```python
from build123d import *

# Parameters (mm, degrees)
SKETCH_1_W             = 60
SKETCH_1_H             = 67.5
EXTRUDE_1_DEPTH        = 6
CUT_EXTRUDE_1_DEPTH    = 47.723254382
HOLE_WIZARD_M5_1_D     = 4.2
HOLE_WIZARD_M5_1_DEPTH = 12.4
HOLE_WIZARD_M5_1_TIP   = 1.2618073


with BuildPart() as part:
    # 草图1 → 凸台-拉伸1 (new, symmetric)
    with BuildSketch(Plane.XY):
        Rectangle(SKETCH_1_W, SKETCH_1_H)
    extrude(amount=EXTRUDE_1_DEPTH, both=True)

    # 草图2 → 切除-拉伸1 (cut, through all)
    with BuildSketch(Plane(origin=(0, 0, -6), x_dir=(-1, 0, 0), z_dir=(0, 0, -1))):
        with BuildLine():
            Line((9.3, -28.75), (9.3, -18.75))
            ThreePointArc((9.3, -18.75), (12, -16.05), (14.7, -18.75))
            Line((14.7, -18.75), (14.7, -28.75))
            ThreePointArc((14.7, -28.75), (12, -31.45), (9.3, -28.75))
        make_face()
        with BuildLine():
            Line((-14.7, -28.75), (-14.7, -18.75))
            ThreePointArc((-14.7, -18.75), (-12, -16.05), (-9.3, -18.75))
            Line((-9.3, -18.75), (-9.3, -28.75))
            ThreePointArc((-9.3, -28.75), (-12, -31.45), (-14.7, -28.75))
        make_face()
        with BuildLine():
            Line((14.7, 5.25), (14.7, -4.75))
            ThreePointArc((14.7, -4.75), (12, -7.45), (9.3, -4.75))
            Line((9.3, -4.75), (9.3, 5.25))
            ThreePointArc((9.3, 5.25), (12, 7.95), (14.7, 5.25))
        make_face()
        with BuildLine():
            Line((-9.3, 5.25), (-9.3, -4.75))
            ThreePointArc((-9.3, -4.75), (-12, -7.45), (-14.7, -4.75))
            Line((-14.7, -4.75), (-14.7, 5.25))
            ThreePointArc((-14.7, 5.25), (-12, 7.95), (-9.3, 5.25))
        make_face()
    extrude(amount=-CUT_EXTRUDE_1_DEPTH, mode=Mode.SUBTRACT)

    # M5 螺纹孔1
    with Locations(Plane(origin=(0, 33.75, 0), x_dir=(1, 0, 0), z_dir=(0, 1, 0))):
        with Locations((-15, 0), (15, 0)):
            Hole(HOLE_WIZARD_M5_1_D / 2, depth=HOLE_WIZARD_M5_1_DEPTH)
            with Locations((0, 0, -(HOLE_WIZARD_M5_1_DEPTH + HOLE_WIZARD_M5_1_TIP / 2))):  # 118° drill point
                Cone(0, HOLE_WIZARD_M5_1_D / 2, HOLE_WIZARD_M5_1_TIP, mode=Mode.SUBTRACT)


solid = part.part
```
Check sheet for the modelled part. Datum: model origin and axes. Units: mm. A direction names the side the tool comes from. Give positions to 0.01 mm unless a question says otherwise; leave off trailing zeros. Write each loop counter-clockwise with the first axis right and the second up, starting at its lowest first coordinate (ties: lowest second). Pieces come first, ordered by that corner, then holes. Notation, with made-up numbers: (74, 9) - (89, 9) arc R21 ccw to (89, 41) - close; hole circle Ø11 at (7, 62.5). An arc over 180 degrees is marked (long way). Answer as a JSON object with one key per item and string values. Group by question number.
1) Thickness scan on probe 1 along X at (y, z) = (-22, 3); probe 2 along Y at (x, z) = (-12, 3.25); probe 3 along Z at (x, y) = (15, 26.25). Record the ranges inside material, lowest first. Write a range as from..to.
2) Sectioned sample at B-B (z = 3.25). Record the cut outline in (x, y).
3) Access from +Z, -Z, +X, -X, +Y, -Y to the whole of each face (thin tool, end or side, straight path). Record for faces 4 (the face through (12.06, 7.95, -0.08)), 5 (the face through (30, 0, 0)), 6 (the face through (-12.9, 27.46, -0.09)).
4) Sectioned sample at C-C (x = -12). Record the cut outline in (y, z), then the cut area to 3 significant figures.
5) Sectioned sample at A-A (y = -20). Record the cut outline in (x, z), then the cut area to 3 significant figures.
6) Release check for a two-part mould opening along Z. For faces 1 (the face through (17.1, 27.46, -0.09)), 2 (the face through (0, 0, -6)), 3 (the face through (-11.94, 7.95, -0.08)) record: pulls with the +Z half, pulls with the -Z half, needs draft (parallel to the pull), parting line crosses it, or undercut.
Geometry results:
{
 "1": {"probe 1": "x = -30..-14.7, -9.3..9.3, 14.7..30", "probe 2": "y = -33.75..-31.45, -16.05..-7.45, 7.95..33.75", "probe 3": "z = -6..-2.1, 2.1..6"},
 "2": {"outline": "(-30, -33.75) - (30, -33.75) - (30, 33.75) - (-30, 33.75) - close; hole (-14.7, -28.75) arc R2.7 ccw to (-9.3, -28.75) - (-9.3, -18.75) arc R2.7 ccw to (-14.7, -18.75) - close; hole (-14.7, -4.75) arc R2.7 ccw to (-9.3, -4.75) - (-9.3, 5.25) arc R2.7 ccw to (-14.7, 5.25) - close; hole (9.3, -28.75) arc R2.7 ccw to (14.7, -28.75) - (14.7, -18.75) arc R2.7 ccw to (9.3, -18.75) - close; hole (9.3, -4.75) arc R2.7 ccw to (14.7, -4.75) - (14.7, 5.25) arc R2.7 ccw to (9.3, 5.25) - close"},
 "3": {"face 4": "+Z, -Z", "face 5": "+Z, -Z, +X, +Y, -Y", "face 6": "+Y"},
 "4": {"outline": "(-33.75, -6) - (-31.45, -6) - (-31.45, 6) - (-33.75, 6) - close; (-16.05, -6) - (-7.45, -6) - (-7.45, 6) - (-16.05, 6) - close; (7.95, -6) - (33.75, -6) - (33.75, 6) - (7.95, 6) - close", "area": "440 mm^2"},
 "5": {"outline": "(-30, -6) - (-14.7, -6) - (-14.7, 6) - (-30, 6) - close; (-9.3, -6) - (9.3, -6) - (9.3, 6) - (-9.3, 6) - close; (14.7, -6) - (30, -6) - (30, 6) - (14.7, 6) - close", "area": "590 mm^2"},
 "6": {"face 1": "undercut", "face 2": "pulls with the -Z half", "face 3": "needs draft"}
}
